Here's how the part is built. I have some questions about the finished solid (model axes, mm). Round coordinates to 2 decimals unless told otherwise and drop trailing zeros. Loops run counter-clockwise (first coordinate to the right, second up) from the corner with the lowest first, then second, coordinate; pieces in that order, holes last. Notation, with made-up numbers: M -22,61 L 7,61 A23 cw 7,90 Z; hole C 27.25,1.25 d2. An arc over 180 degrees is marked long. Answer as a JSON object with one key per item and string values.
from build123d import *

# Parameters (mm, degrees)
SKETCH1_R           = 2
BOSS_EXTRUDE1_DEPTH = 1


with BuildPart() as part:
    # Sketch1 → Boss-Extrude1 (new body)
    with BuildSketch(Plane.XY):
        Polygon((-40, 40), (40, 40), (40, 32), (50, 32), (50, -32), (40, -32), (40, -40), (-40, -40), (-40, -32), (-50, -32), (-50, 32), (-40, 32), align=None)
        with Locations((-25, 36)):
            Circle(SKETCH1_R, mode=Mode.SUBTRACT)
        with Locations((-25, -36)):
            Circle(SKETCH1_R, mode=Mode.SUBTRACT)
        with Locations((25, 36)):
            Circle(SKETCH1_R, mode=Mode.SUBTRACT)
        with Locations((25, -36)):
            Circle(SKETCH1_R, mode=Mode.SUBTRACT)
    extrude(amount=BOSS_EXTRUDE1_DEPTH)


solid = part.part
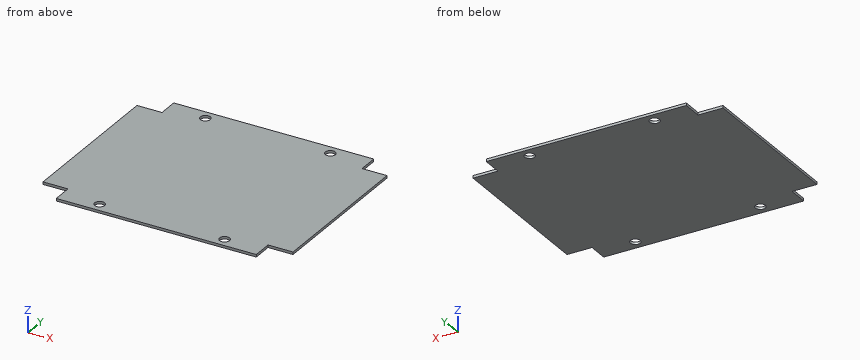
Item 1: I want a section at C-C on z = 0.5. List the corners of the cut face in (x, y) for me, plus the area to 3 significant figures.
Solution:
{"outline": "M -50,-32 L -40,-32 L -40,-40 L 40,-40 L 40,-32 L 50,-32 L 50,32 L 40,32 L 40,40 L -40,40 L -40,32 L -50,32 Z; hole C -25,-36 d4; hole C -25,36 d4; hole C 25,-36 d4; hole C 25,36 d4", "area": "7,630 mm2"}
Item 2: I want a section at B-B on y = 36. List the corners of the cut face in (x, z) for me.
Solution:
{"outline": "M -40,0 L -27,0 L -27,1 L -40,1 Z; M -23,0 L 23,0 L 23,1 L -23,1 Z; M 27,0 L 40,0 L 40,1 L 27,1 Z"}
Item 3: If I drill on L1, parallel to Y at x = 25, z = 0.5, over which ranges is the centre line in solid material (lowest first)? Write a range as from..to.
Solution:
{"L1": "y = -40..-38, -34..34, 38..40"}
Item 4: For P1, Ø0.5, axis at y = -36.5, z = 0.5, coming from the -X side; P2, Ø2.5, axis at x = -25, y = 36, coming from the -Z side, each with a flat end and sliding along its axis, tell me the tip position at first contact or that it passes through.
Solution:
{"P1": "stops at x = -40", "P2": "passes through"}
Item 5: I want a section at A-A on x = 25. List the corners of the cut face in (y, z) for me, plus the area to 3 significant figures.
Solution:
{"outline": "M -40,0 L -38,0 L -38,1 L -40,1 Z; M -34,0 L 34,0 L 34,1 L -34,1 Z; M 38,0 L 40,0 L 40,1 L 38,1 Z", "area": "72.0 mm2"}
